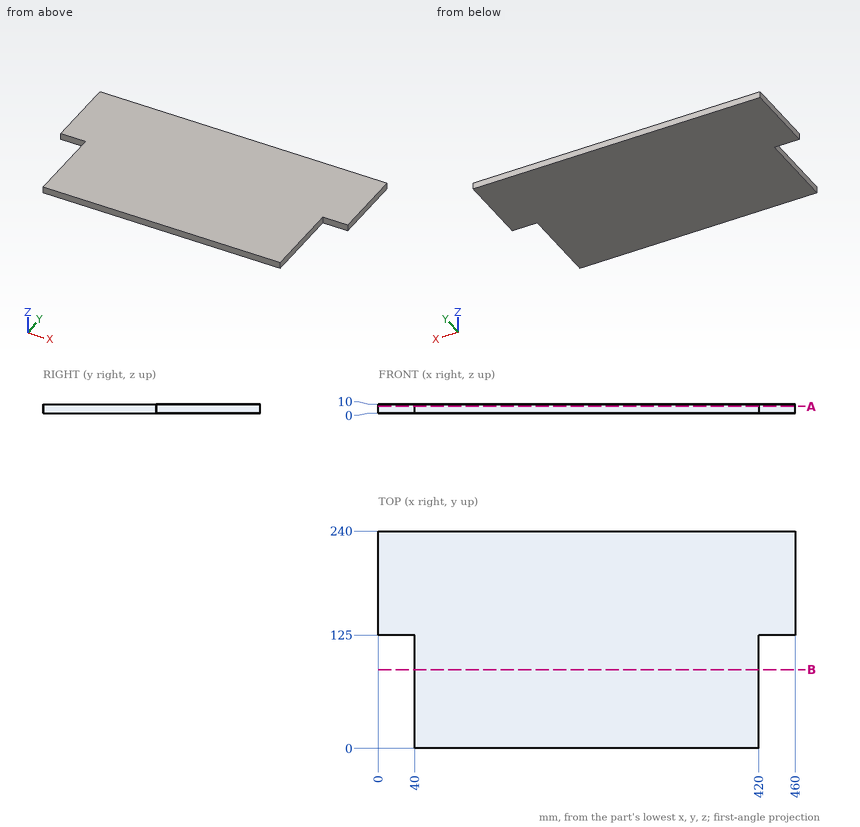
Could you check a few things on this drawing? It's one solid part, dimensions in mm from its lowest x, y, z. Give positions to 0.01 mm unless a question says otherwise; leave off trailing zeros. Order: outer loops, then holes, each group sorted by start corner. A loop starts at its lowest first (then second) coordinate and runs counter-clockwise, first axis right, second up. Notation, with made-up numbers: (-24, 33) - (35, 33) arc R9 ccw to (35, 40) - close; hole circle Ø5 at (52, 6.5). An arc over 180 degrees is marked (long way). One line per question, with ' | ' between items. Start each with the question number.
Item 1: I need wall thicknesses on probe 1 along X at (y, z) = (82, 1.5); probe 2 along Y at (x, z) = (424.5, 6). Which ranges of each line are inside material? Lowest first, please. Write a range as [from, to].
Item 2: I'm going to push flat-ended pins straight in: pin 1 Ø6 at (y, z) = (206, 3.5) entering from -X; pin 2 Ø3 at (x, z) = (434.5, 3.5) entering from -Y; pin 3 Ø5 at (y, z) = (54, 4) entering from -X. Where does each tip first touch, or does it pass through?
Item 3: I want a section at A-A on z = 7.5. Write out the boundary of the cut face in (x, y), then the cut area to 3 significant figures.
Item 4: I want a section at B-B on y = 87. Write out the boundary of the cut face in (x, z), then the cut area to 3 significant figures.
Verdict:
1) probe 1: [40, 420] | probe 2: [125, 240]
2) pin 1: x = 0 | pin 2: y = 125 | pin 3: x = 40
3) outline: (0, 125) - (40, 125) - (40, 0) - (420, 0) - (420, 125) - (460, 125) - (460, 240) - (0, 240) - close | area: 100,000 mm^2
4) outline: (40, 0) - (420, 0) - (420, 10) - (40, 10) - close | area: 3,800 mm^2
